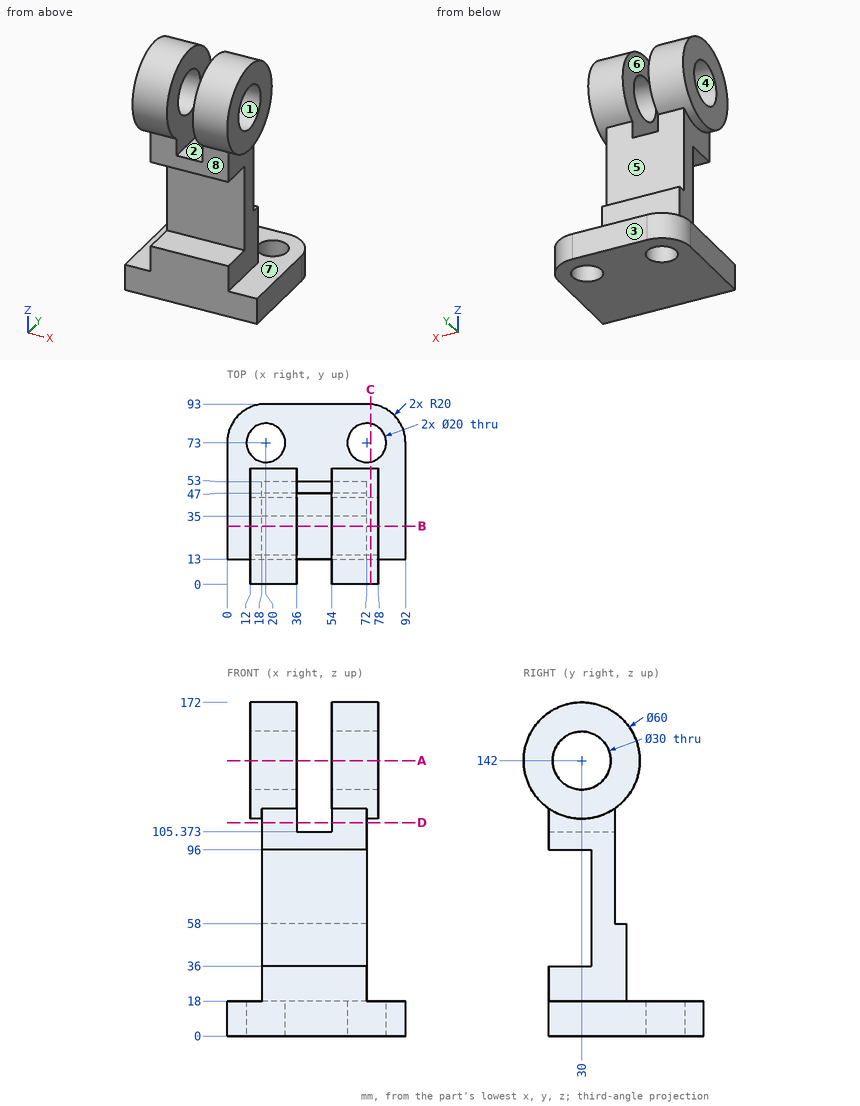
Design review of the part shown in the three views and the two pictorial views. Dimensions are in mm from the part's minimum x, y and z. A direction names the side the tool comes from. Round coordinates to 2 decimals unless told otherwise and drop trailing zeros. Loops run counter-clockwise (first coordinate to the right, second up) from the corner with the lowest first, then second, coordinate; pieces in that order, holes last. Notation, with made-up numbers: (41, 45.5) -> (46, 45.5) arc R19 cw to (46, 58.5) -> close; hole circle Ø11 at (-40, 68.5). An arc over 180 degrees is marked (long way). Use one line per item in the form item = value. Start each with the question number.
Q1. We need section D-D on z = 110. Give the boundary of the cut face in (x, y).
Q2. We need section B-B on y = 30. Give the boundary of the cut face in (x, z).
Q3. Draft analysis for pull direction Y (two halves, no side actions). For the marked faces 1, 2, 3 and 4, state which applies: +Y half, -Y half, draft (parallel to the pull), parting line (faces both ways), or undercut.
Q4. Machinability: for the marked faces 5, 6, 7 and 8, which of the approach directions +Z, -Z, +X, -X, +Y, -Y give a long, thin tool a straight path to every point of the face, cutting with its end or side? Answer none if there is none.
Q5. For pin 1 Ø6.5 at (x, y) = (38.5, 50.5) entering from +Z (1 decimal); pin 2 Ø1 at (x, y) = (55.5, 48) entering from +Z; pin 3 Ø18 at (y, z) = (38.5, 150.5) entering from -X; pin 4 Ø18 at (x, y) = (72, 73) entering from -Z, all flat-tipped, find the tip position at first contact; note any pin that passes through.
Q6. We need section C-C on x = 74. Give the boundary of the cut face in (y, z), then the cut area to 3 significant figures.
Q7. Wall thickness on line 1 along Z through (x, y) = (68, 30); line 2 along Z through (x, y) = (48, 17.5); line 3 along X through (y, z) = (40, 130): over which ranges is each line inside the solid? List them lowest first. Write a range as [from, to].
Q8. We need section A-A on z = 142. Give the boundary of the cut face in (x, y), then the cut area to 3 significant figures.
Calculated:
q1.outline = (18, 13) -> (36, 13) -> (36, 47) -> (18, 47) -> close; (54, 13) -> (72, 13) -> (72, 47) -> (54, 47) -> close
q2.outline = (0, 0) -> (92, 0) -> (92, 18) -> (72, 18) -> (72, 36) -> (18, 36) -> (18, 18) -> (0, 18) -> close; (12, 112) -> (18, 112) -> (18, 96) -> (72, 96) -> (72, 112) -> (78, 112) -> (78, 127) -> (54, 127) -> (54, 105.37) -> (36, 105.37) -> (36, 127) -> (12, 127) -> close; (12, 157) -> (36, 157) -> (36, 172) -> (12, 172) -> close; (54, 157) -> (78, 157) -> (78, 172) -> (54, 172) -> close
q3.face_1 = undercut
q3.face_2 = draft
q3.face_3 = +Y half
q3.face_4 = undercut
q4.face_5 = +X, -X, +Y
q4.face_6 = +Z, +Y, -Y
q4.face_7 = +Y
q4.face_8 = -Z, +X, -X, -Y
q5.pin_1 = 165.7
q5.pin_2 = 166.37
q5.pin_3 = 12
q5.pin_4 = through
q6.outline = circle Ø60 at (30, 142); (13, 0) -> (63.2, 0) -> (63.2, 18) -> (13, 18) -> close; (82.8, 0) -> (92.9, 0) -> (92.9, 18) -> (82.8, 18) -> close; hole circle Ø30 at (30, 142)
q6.area = 3,210 mm²
q7.line_1 = [0, 36], [96, 127], [157, 172]
q7.line_2 = [0, 36], [96, 105.37]
q7.line_3 = [12, 36], [54, 78]
q8.outline = (12, 0) -> (36, 0) -> (36, 15) -> (12, 15) -> close; (12, 45) -> (36, 45) -> (36, 60) -> (12, 60) -> close; (54, 0) -> (78, 0) -> (78, 15) -> (54, 15) -> close; (54, 45) -> (78, 45) -> (78, 60) -> (54, 60) -> close
q8.area = 1,440 mm²
